Check sheet for the drawn part. Datum: minimum x, y, z corner. Units: mm. A direction names the side the tool comes from. Round coordinates to 2 decimals unless told otherwise and drop trailing zeros. Write each loop counter-clockwise with the first axis right and the second up, starting at its lowest first coordinate (ties: lowest second). Pieces come first, ordered by that corner, then holes.
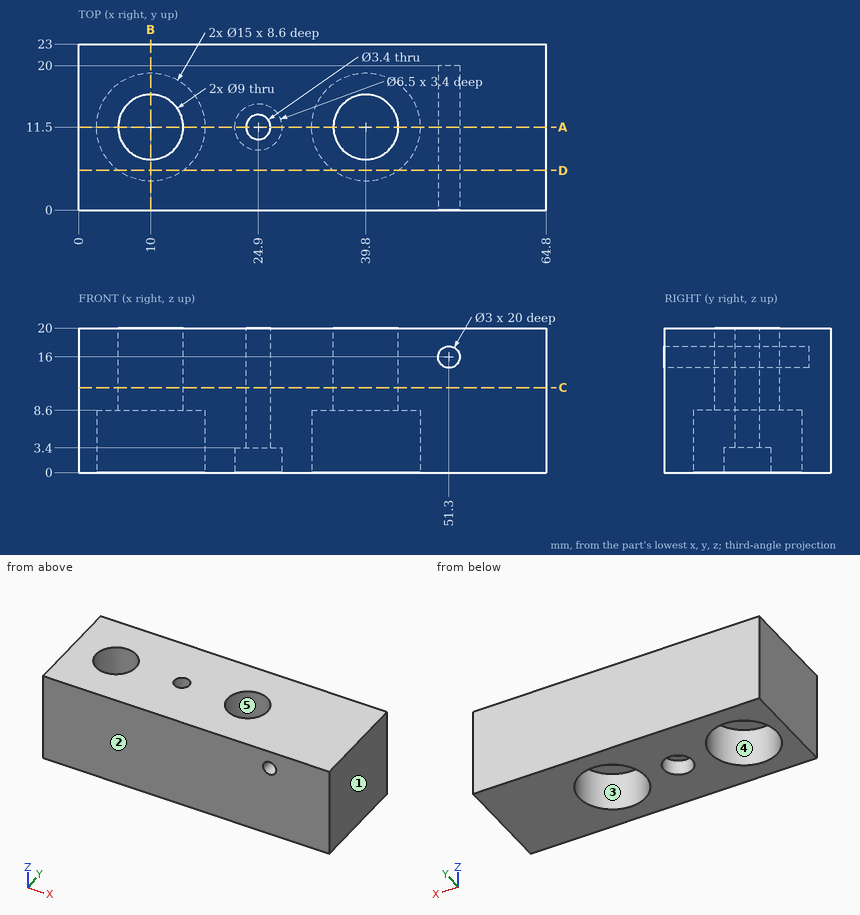
Q1. Sectioned sample at D-D (y = 5.5). Enter the section's corners in (x, z), plus the area to 3 significant figures.
Recorded:
outline: (0, 0) - (5.5, 0) - (5.5, 8.6) - (14.5, 8.6) - (14.5, 0) - (35.3, 0) - (35.3, 8.6) - (44.3, 8.6) - (44.3, 0) - (64.8, 0) - (64.8, 20) - (0, 20) - close; hole circle Ø3 at (51.3, 16)
area: 1,130 mm2
Q2. Sectioned sample at C-C (z = 11.75). Enter the section's corners in (x, y).
Recorded:
outline: (0, 0) - (64.8, 0) - (64.8, 23) - (0, 23) - close; hole circle Ø9 at (10, 11.5); hole circle Ø3.4 at (24.9, 11.5); hole circle Ø9 at (39.8, 11.5)
Q3. Sectioned sample at B-B (x = 10). Enter the section's corners in (y, z), plus the area to 3 significant figures.
Recorded:
outline: (0, 0) - (4, 0) - (4, 8.6) - (7, 8.6) - (7, 20) - (0, 20) - close; (16, 8.6) - (19, 8.6) - (19, 0) - (23, 0) - (23, 20) - (16, 20) - close
area: 228 mm2
Q4. Material ranges on line 1 along Y through (x, z) = (39.8, 3.25); line 2 along Y through (x, z) = (40, 17); line 3 along X through (y, z) = (10, 18.5), recorded low to high.
Recorded:
line 1: y = 0 to 4, 19 to 23
line 2: y = 0 to 7, 16 to 23
line 3: x = 0 to 5.76, 14.24 to 24.1, 25.7 to 35.56, 44.04 to 64.8
Q5. Tool access check on the marked faces 4 and 5. Record the directions out of +Z, -Z, +X, -X, +Y, -Y that give a thin tool (end or side, any length) a straight path to the whole face; none if there is none.
Recorded:
face 4: -Z
face 5: +Z, -Z
Q6. Depth check by flat-ended pin: P1, Ø12, axis at x = 39.8, y = 11.5, coming from the -Z side; P2, Ø7, axis at x = 39.8, y = 11.5, coming from the +Z side. Enter the tip coordinate at first touch or a pass-through.
Recorded:
P1: stops at z = 8.6
P2: passes through
Q7. Release check for a two-part mould opening along X. For the marked faces 1, 2 and 3 record: released by +X, released by -X, zero draft, split by the parting line, or undercut.
Recorded:
face 1: released by +X
face 2: zero draft
face 3: undercut
Q8. Sectioned sample at A-A (y = 11.5). Give the number of separate pieces and of enclosed holes in the cut face, plus the area to 3 significant figures.
Recorded:
separate pieces: 4
enclosed holes: 1
area: 747 mm2
